```python
from build123d import *

# Parameters (mm, degrees)
SKETCH_1_W          = 480
SKETCH_1_H          = 60
EXTRUDE_1_DEPTH     = 16
SKETCH_2_W          = 200
SKETCH_2_H          = 60
CUT_EXTRUDE_1_DEPTH = 6
SKETCH_3_W          = 12
SKETCH_3_H          = 60
CUT_EXTRUDE_2_DEPTH = 6
SKETCH_4_R          = 2.1
SKETCH_4_R_2        = 2.5
CUT_EXTRUDE_3_DEPTH = 322.959006961
SKETCH_5_W          = 80
SKETCH_5_H          = 60
CUT_EXTRUDE_4_DEPTH = 14


with BuildPart() as part:
    # 草图1 → 凸台-拉伸1 (new body)
    with BuildSketch(Plane.XY):
        with Locations((80.192307692, -2.163461538)):
            Rectangle(SKETCH_1_W, SKETCH_1_H)
    extrude(amount=EXTRUDE_1_DEPTH)

    # 草图2 → 切除-拉伸1 (cut)
    with BuildSketch(Plane.XY.offset(16)):
        with Locations((-59.807692308, -2.163461538)):
            Rectangle(SKETCH_2_W, SKETCH_2_H)
    extrude(amount=-CUT_EXTRUDE_1_DEPTH, mode=Mode.SUBTRACT)

    # 草图3 → 切除-拉伸2 (cut)
    with BuildSketch(Plane.XY.offset(16)):
        with Locations((106.192307692, -2.163461538)):
            Rectangle(SKETCH_3_W, SKETCH_3_H)
        with Locations((156.192307692, -2.163461538)):
            Rectangle(SKETCH_3_W, SKETCH_3_H)
    extrude(amount=-CUT_EXTRUDE_2_DEPTH, mode=Mode.SUBTRACT)

    # 草图4 → 切除-拉伸3 (cut, through all)
    with BuildSketch(Plane.XY.offset(10)):
        with Locations((-134.807692308, 17.836538462)):
            Circle(SKETCH_4_R)
        with Locations((-134.807692308, -22.163461538)):
            Circle(SKETCH_4_R)
        with Locations((25.192307692, 17.836538462)):
            Circle(SKETCH_4_R)
        with Locations((25.192307692, -22.163461538)):
            Circle(SKETCH_4_R)
        with Locations((106.192307692, 18.336538462)):
            Circle(SKETCH_4_R)
        with Locations((106.192307692, -22.663461538)):
            Circle(SKETCH_4_R)
        with Locations((156.192307692, 18.336538462)):
            Circle(SKETCH_4_R)
        with Locations((156.192307692, -22.663461538)):
            Circle(SKETCH_4_R)
        with Locations((106.192307692, -2.163461538)):
            Circle(SKETCH_4_R_2)
        with Locations((156.192307692, -2.163461538)):
            Circle(SKETCH_4_R_2)
    extrude(amount=-CUT_EXTRUDE_3_DEPTH, mode=Mode.SUBTRACT)

    # 草图5 → 切除-拉伸4 (cut)
    with BuildSketch(Plane.XY.offset(16)):
        with Locations((247.192307692, -2.163461538)):
            Rectangle(SKETCH_5_W, SKETCH_5_H)
    extrude(amount=-CUT_EXTRUDE_4_DEPTH, mode=Mode.SUBTRACT)


solid = part.part
```
Verification items for the finished model (mm, model axes). A direction names the side the tool comes from. Coordinates: 2 decimals unless noted, no trailing zeros. Write each loop counter-clockwise with the first axis right and the second up, starting at its lowest first coordinate (ties: lowest second). Pieces come first, ordered by that corner, then holes. Notation, with made-up numbers: (76.25, 70) - (127.25, 70) arc R31 ccw to (127.25, 99) - close; hole circle Ø3 at (2, 4.25). An arc over 180 degrees is marked (long way). One line per question, with ' | ' between items. Start each with the question number.
1. Access from +Z, -Z, +X, -X, +Y, -Y to the whole of each face (thin tool, end or side, straight path). Record for faces 1 (the flat face through (184, -2, 16)), 2 (the flat face through (153, -2, 10)), 3 (the flat face through (-61, -2, 10)).
2. Section check C-C (x = 212.5). Enter the section's corners in (y, z).
3. Gauge pin test, flat ends, axial feed: P1, Ø6.5, axis at x = 106.19, y = 18.34, coming from the +Z side; P2, Ø12, axis at x = 272, y = -17.5, coming from the -Z side; P3, Ø6.5, axis at y = 10, z = 13.5, coming from the -X side; P4, Ø3.5, axis at x = 156.19, y = -22.66, coming from the +Z side. Record the tip position at first contact, or that the pin passes through.
4. Draft check along X on faces 4 (the flat face through (77, -32.163, 6)), 5 (the flat face through (287.192, -3, 9)), 6 (the flat face through (320.192, -3, 8)). Enter one of: released by +X, released by -X, zero draft, split by the parting line, or undercut.
5. Section check A-A (z = 13). Enter the section's corners in (x, y), plus the area to 3 significant figures.
6. Material ranges on line 1 along X through (y, z) = (-6, 12.5); line 2 along X through (y, z) = (-1.5, 1.75); line 3 along X through (y, z) = (4, 5.5), recorded low to high.
7. Section check B-B (y = 7). Enter the section's corners in (x, z), plus the area to 3 significant figures.
Computed values:
1) face 1: +Z, +X, -X, +Y, -Y | face 2: +Z, +Y, -Y | face 3: +Z, -X, +Y, -Y
2) outline: (-32.16, 0) - (27.84, 0) - (27.84, 2) - (-32.16, 2) - close
3) P1: z = 10 | P2: z = 0 | P3: x = 40.19 | P4: through
4) face 4: zero draft | face 5: undercut | face 6: released by +X
5) outline: (40.19, -32.16) - (100.19, -32.16) - (100.19, 27.84) - (40.19, 27.84) - close; (112.19, -32.16) - (150.19, -32.16) - (150.19, 27.84) - (112.19, 27.84) - close; (162.19, -32.16) - (207.19, -32.16) - (207.19, 27.84) - (162.19, 27.84) - close; (287.19, -32.16) - (320.19, -32.16) - (320.19, 27.84) - (287.19, 27.84) - close | area: 10,600 mm²
6) line 1: 40.19 to 100.19, 112.19 to 150.19, 162.19 to 207.19, 287.19 to 320.19 | line 2: -159.81 to 103.78, 108.6 to 153.78, 158.6 to 320.19 | line 3: -159.81 to 207.19, 287.19 to 320.19
7) outline: (-159.81, 0) - (320.19, 0) - (320.19, 16) - (287.19, 16) - (287.19, 2) - (207.19, 2) - (207.19, 16) - (162.19, 16) - (162.19, 10) - (150.19, 10) - (150.19, 16) - (112.19, 16) - (112.19, 10) - (100.19, 10) - (100.19, 16) - (40.19, 16) - (40.19, 10) - (-159.81, 10) - close | area: 5,220 mm²
